Geometry: final body of the model. Coordinates: model frame, mm. A direction names the side the tool comes from. Coordinates: 2 decimals unless noted, no trailing zeros. Order: outer loops, then holes, each group sorted by start corner. A loop starts at its lowest first (then second) coordinate and runs counter-clockwise, first axis right, second up. Notation, with made-up numbers: M 65.5,-1.75 L 73.5,-1.75 A21 ccw 73.5,4.25 Z; hole C -28.75,9.5 d1. An arc over 180 degrees is marked long. One line per question, with ' | ' between items.
from build123d import *

# Parameters (mm, degrees)
SKETCH2_W           = 8
SKETCH2_H           = 8
BOSS_EXTRUDE1_DEPTH = 15
CHAMFER1_SIZE       = 2


with BuildPart() as part:
    # Sketch1 → Revolve1 (revolve)
    with BuildSketch(Plane.XY, mode=Mode.PRIVATE) as revolve1_sk:
        Polygon((0, 0), (0, 5), (12, 5), (12, 7.845), (80, 7.845), (80, 0), align=None)
    revolve(revolve1_sk.sketch.rotate(Axis((0, 0, 0), (1, 0, 0)), 90), axis=Axis((0, 0, 0), (1, 0, 0)))

    # Sketch2 → Boss-Extrude1 (add)
    with BuildSketch(Plane(origin=(80, 0, 0), x_dir=(0, 0, -1), z_dir=(1, 0, 0))):
        Rectangle(SKETCH2_W, SKETCH2_H)
    extrude(amount=BOSS_EXTRUDE1_DEPTH)

    # Chamfer1
    chamfer1_edges = [part.edges().sort_by_distance(p)[0] for p in [
        (0, 0, -5),
    ]]
    chamfer(chamfer1_edges, length=CHAMFER1_SIZE)


solid = part.part
1. Access query for faces 1 (the face through (87, 4, 0)), 2 (the face through (87, 0, 4)), 3 (the face through (12, 2, -5)), 4 (the face through (87, 0, -4)). Directions: +Z, -Z, +X, -X, +Y, -Y. A direction counts if a zero-diameter tool reaches every point of the face in a straight line with its end or side. Return the directions, or none.
Response values:
face 1: +Z, -Z, +X, +Y | face 2: +Z, +X, +Y, -Y | face 3: -X | face 4: -Z, +X, +Y, -Y
2. Material intervals for line 1 (Y direction, x = 85.5, z = -0.75); line 2 (X direction, y = 5.5, z = -1.75); line 3 (Z direction, x = 64.5, y = 0.25), sorted ascending. Write a range as [from, to].
Response values:
line 1: y = [-4, 4] | line 2: x = [12, 80] | line 3: z = [-7.84, 7.84]
3. Section C-C, the plane x = 55. Output: boundary loops of the cut face in (y, z) (3 decimals).
Response values:
outline: C 0,0 d15.69
4. Pin query (flat end, axial travel): P1, Ø9, axis at x = 87, z = 2, coming from the +Y side; P2, Ø2, axis at x = 65.5, z = -1.5, coming from the +Y side; P3, Ø1.5, axis at y = 2, z = -5.5, coming from the -X side. Return the tip coordinate at first contact, or that it passes through.
Response values:
P1: stops at y = 4 | P2: stops at y = 7.83 | P3: stops at x = 12
5. Section A-A, the plane y = 0. Output: boundary loops of the cut face in (x, z) (3 decimals), and give its area (3 significant figures).
Response values:
outline: M 0,-3 L 2,-5 L 12,-5 L 12,-7.845 L 80,-7.845 L 80,-4 L 95,-4 L 95,4 L 80,4 L 80,7.845 L 12,7.845 L 12,5 L 2,5 L 0,3 Z | area: 1,300 mm^2
